from build123d import *

# Parameters (mm, degrees)
SKETCH1_R           = 50
BOSS_EXTRUDE1_DEPTH = 40
SKETCH2_R           = 16.25
CUT_EXTRUDE1_DEPTH  = 150
SKETCH10_R          = 100
CUT_EXTRUDE5_DEPTH  = 20
SKETCH11_R          = 30
SKETCH11_R_2        = 16.25
BOSS_EXTRUDE2_DEPTH = 20
SKETCH12_R          = 130
CUT_EXTRUDE7_DEPTH  = 30


with BuildPart() as part:
    # Sketch1 → Boss-Extrude1 (new, symmetric)
    with BuildSketch(Plane.XY):
        Circle(SKETCH1_R)
    extrude(amount=BOSS_EXTRUDE1_DEPTH, both=True)

    # Sketch2 → Cut-Extrude1 (cut)
    with BuildSketch(Plane.XY.offset(40)):
        Circle(SKETCH2_R)
    extrude(amount=-CUT_EXTRUDE1_DEPTH, mode=Mode.SUBTRACT)

    # Sketch4 → Cut-Revolve1 (revolve, cut)
    with BuildSketch(Plane(origin=(0, 0, 0), x_dir=(0, 0, -1), z_dir=(1, 0, 0)), mode=Mode.PRIVATE) as cut_revolve1_sk:
        Polygon((-40, 50), (-36.6, 50), (-33.604349764, 41.3), (-26.395650236, 41.3), (-23.4, 50), (-21.6, 50), (-18.604349764, 41.3), (-11.395650236, 41.3), (-8.4, 50), (-6.6, 50), (-3.604349764, 41.3), (3.604349764, 41.3), (6.6, 50), (10, 50), (10, 161.050459045), (-40, 161.050459045), align=None)
    revolve(cut_revolve1_sk.sketch.rotate(Axis((0, 0, 0), (0, 0, -1)), 90), axis=Axis((0, 0, 0), (0, 0, -1)), mode=Mode.SUBTRACT)

    # Sketch10 → Cut-Extrude5 (cut)
    with BuildSketch(Plane(origin=(0, 0, -40), x_dir=(-1, 0, 0), z_dir=(0, 0, -1))):
        Circle(SKETCH10_R)
    extrude(amount=-CUT_EXTRUDE5_DEPTH, mode=Mode.SUBTRACT)

    # Sketch11 → Boss-Extrude2 (add)
    with BuildSketch(Plane(origin=(0, 0, -20), x_dir=(-1, 0, 0), z_dir=(0, 0, -1))):
        Circle(SKETCH11_R)
        with Locations(Location((0, 0, 0), (0, 0, 180))):
            Circle(SKETCH11_R_2, mode=Mode.SUBTRACT)
    extrude(amount=BOSS_EXTRUDE2_DEPTH)

    # Sketch12 → Cut-Extrude7 (cut)
    with BuildSketch(Plane(origin=(0, 0, -40), x_dir=(-1, 0, 0), z_dir=(0, 0, -1))):
        Circle(SKETCH12_R)
    extrude(amount=-CUT_EXTRUDE7_DEPTH, mode=Mode.SUBTRACT)


solid = part.part
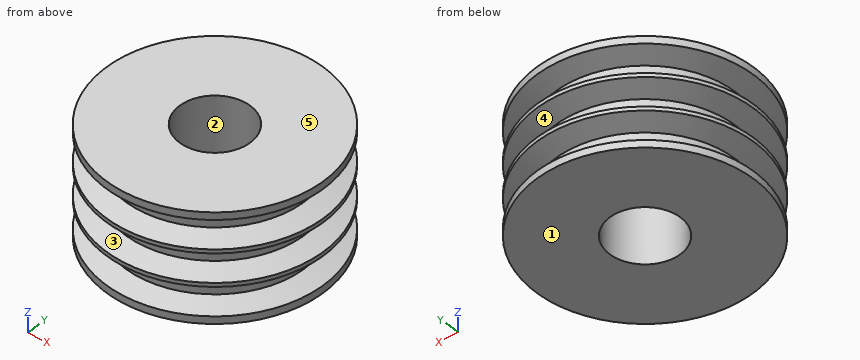
Source: CAD feature listing. Evaluate the final solid. Frame: model axes, mm. Face numbers are marked on the shaded views. A direction names the side the tool comes from. Give positions to 0.01 mm unless a question says otherwise; leave off trailing zeros. Order: outer loops, then holes, each group sorted by start corner. A loop starts at its lowest first (then second) coordinate and runs counter-clockwise, first axis right, second up. Notation, with made-up numbers: (6.5, 65.25) -> (58.5, 65.25) arc R12 ccw to (58.5, 75.25) -> close; hole circle Ø9 at (-39, 59.5). An arc over 180 degrees is marked (long way). Use a Markdown table: item, result.
1) Ray query, line 1 along Z through (x, y) = (-13, 44.5); line 2 along Z through (x, y) = (13.5, -40.5); line 3 along X through (y, z) = (-31, 8). Return the intervals inside material, ascending. Write a range as [from, to].
Answer list:
| item | result |
|---|---|
| line 1 | [-10, -5.35], [5.35, 9.65], [20.35, 24.65], [35.35, 40] |
| line 2 | [-10, -4.08], [4.08, 10.92], [19.08, 25.92], [34.08, 40] |
| line 3 | [-39.23, 39.23] |
2) Mould query, pull axis X, two halves, no side actions, for the marked faces 1, 2 and 3. Classes: +X half, -X half, draft (parallel to the pull), parting line (faces both ways), or undercut.
Answer list:
| item | result |
|---|---|
| face 1 | draft |
| face 2 | undercut |
| face 3 | parting line |
3) Section query D-D, the plane x = 44. Count the separate pieces of the cut face and the enclosed holes in it, then the cut area to 3 significant figures.
Answer list:
| item | result |
|---|---|
| separate pieces | 4 |
| enclosed holes | 0 |
| area | 881 mm² |
4) Contact query for flat-ended pins moving along their axis: P1, Ø6, axis at x = -35.5, z = 30.5, coming from the +Y side; P2, Ø6, axis at y = 36, z = 1, coming from the -X side; P3, Ø4, axis at y = -30.5, z = 1.5, coming from the +X side. Output: stop coordinate, or through.
Answer list:
| item | result |
|---|---|
| P1 | y = 25.48 |
| P2 | x = -24.83 |
| P3 | x = 29.89 |
5) Reachability of the marked faces 4 and 5 from +Z, -Z, +X, -X, +Y, -Y: full face, straight path, thin tool, end or side. Return the list, or none.
Answer list:
| item | result |
|---|---|
| face 4 | none |
| face 5 | +Z, +X, -X, +Y, -Y |
6) Section query C-C, the plane z = 32. Return the cut outline in (x, y), then the cut area to 3 significant figures.
Answer list:
| item | result |
|---|---|
| outline | circle Ø82.6 at (0, 0); hole circle Ø32.5 at (0, 0) |
| area | 4,530 mm² |
